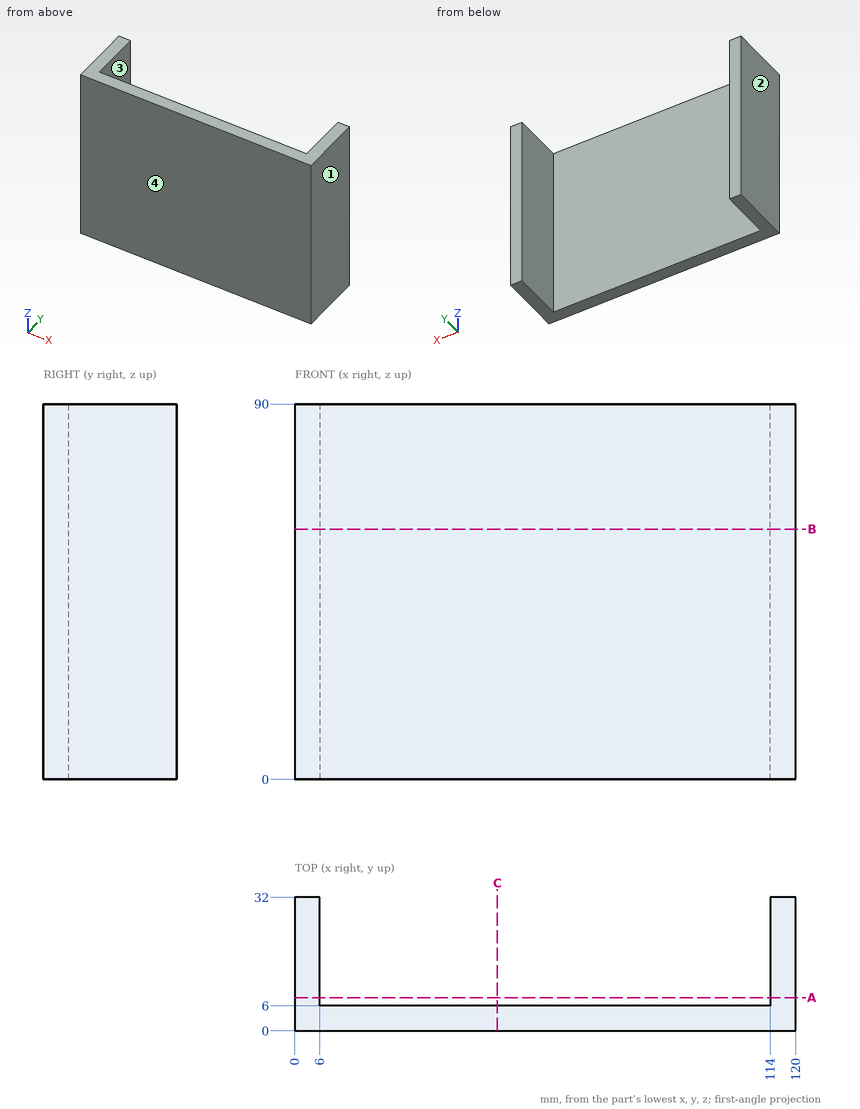
Study the drawing (mm; zero at the part's minimum x, y, z) and answer. Round coordinates to 2 decimals unless told otherwise and drop trailing zeros. Write each loop counter-clockwise with the first axis right and the second up, starting at its lowest first coordinate (ties: lowest second). Pieces come first, ordered by that corner, then holes. Notation, with made-up numbers: (80, 4) -> (133, 4) arc R11 cw to (133, 16) -> close; hole circle Ø9 at (-10, 89). An arc over 180 degrees is marked (long way). Write each question's results on one line, items separated by ' | '.
Item 1: A cutting plane is placed at B-B, the plane z = 60. Determine the outline of the cut face in (x, y), plus the area to 3 significant figures.
Result set:
outline: (0, 0) -> (120, 0) -> (120, 32) -> (114, 32) -> (114, 6) -> (6, 6) -> (6, 32) -> (0, 32) -> close | area: 1,030 mm^2
Item 2: Find the intervals of material crossed by line 1 along X through (y, z) = (10, 44); line 2 along Y through (x, z) = (113, 8), in increasing order. Write a range as [from, to].
Result set:
line 1: [0, 6], [114, 120] | line 2: [0, 6]
Item 3: A cutting plane is placed at C-C, the plane x = 48.5. Determine the outline of the cut face in (y, z).
Result set:
outline: (0, 0) -> (6, 0) -> (6, 90) -> (0, 90) -> close
Item 4: A cutting plane is placed at A-A, the plane y = 8. Determine the outline of the cut face in (x, z).
Result set:
outline: (0, 0) -> (6, 0) -> (6, 90) -> (0, 90) -> close; (114, 0) -> (120, 0) -> (120, 90) -> (114, 90) -> close
Item 5: The mould has two halves that part along X. Classify the marked faces 1, 2, 3 and 4: +X half, -X half, draft (parallel to the pull), parting line (faces both ways), or undercut.
Result set:
face 1: +X half | face 2: -X half | face 3: undercut | face 4: draft
Item 6: A flat-ended cylindrical pin translates along its axis: P1, Ø1.5, axis at x = 72, z = 47.5, coming from the +Y side. Find the tip coordinate at first contact, or state that the pin passes through.
Result set:
P1: y = 6
